```python
from build123d import *

# Parameters (mm, degrees)
SKETCH1_R             = 1.95
BOSS_EXTRUDE1_DEPTH   = 6
M2_TAPPED_HOLE2_D     = 1.6
M2_TAPPED_HOLE2_DEPTH = 6
M2_TAPPED_HOLE2_TIP   = 572.957422794


with BuildPart() as part:
    # Sketch1 → Boss-Extrude1 (new body)
    with BuildSketch(Plane(origin=(0, 0, 0), x_dir=(1, 0, 0), z_dir=(0, 1, 0))):
        Polygon((-6.315, 5.815), (-5.815, 6.315), (5.815, 6.315), (6.315, 5.815), (6.315, -5.815), (5.815, -6.315), (-5.815, -6.315), (-6.315, -5.815), align=None)
        with Locations(Location((0, 0, 0), (0, 0, 270))):
            Circle(SKETCH1_R, mode=Mode.SUBTRACT)
    extrude(amount=BOSS_EXTRUDE1_DEPTH)

    # M2 Tapped Hole2
    with Locations(Plane(origin=(0, 6, 0), x_dir=(-1, 0, 0), z_dir=(0, 1, 0))):
        with Locations((4.25, -4.25), (-4.25, -4.25), (-4.25, 4.25), (4.25, 4.25)):
            Hole(M2_TAPPED_HOLE2_D / 2, depth=M2_TAPPED_HOLE2_DEPTH)
            with Locations((0, 0, -(M2_TAPPED_HOLE2_DEPTH + M2_TAPPED_HOLE2_TIP / 2))):  # 0.16° drill point
                Cone(0, M2_TAPPED_HOLE2_D / 2, M2_TAPPED_HOLE2_TIP, mode=Mode.SUBTRACT)


solid = part.part
```
Can you work these out from the model? Positions are in its coordinate system, mm. Round coordinates to 2 decimals unless told otherwise and drop trailing zeros. Loops run counter-clockwise (first coordinate to the right, second up) from the corner with the lowest first, then second, coordinate; pieces in that order, holes last. Notation, with made-up numbers: M 31,-25 L 66,-25 A26 cw 66,10 Z; hole C 66,67 d1. An arc over 180 degrees is marked long. Write item = value, one per line. Start each with the question number.
(1) Suppose I cut it at B-B on z = 0. Write out the boundary of the cut face in (x, y) (3 decimals).
(2) I need wall thicknesses on line 1 along X through (y, z) = (1.6, -4.25) (3 decimals); line 2 along X through (y, z) = (2.2, -4.75) (1 decimal). Which ranges of each line are inside material? Lowest first, please.
(3) Suppose I cut it at A-A on x = 0. Write out the boundary of the cut face in (y, z) (3 decimals).
(4) Suppose I cut it at C-C on y = 3.35. Write out the boundary of the cut face in (x, z) (3 decimals), plus the area to 3 significant figures.
(5) Suppose I cut it at D-D on z = -4.25. Write out the boundary of the cut face in (x, y) (3 decimals), plus the area to 3 significant figures.
(6) If we mould it in two halves opening along X, with no side actions, what happens to faces 1 (the face through (1.5, 0, -1.5)), 2 (the face through (-4.42, 2.96, -5.03)), 3 (the face through (6.315, 3, 0))? For each: released by +X, released by -X, zero draft, split by the parting line, or undercut.
Answer block:
q1.outline = M -6.315,0 L -1.95,0 L -1.95,6 L -6.315,6 Z; M 1.95,0 L 6.315,0 L 6.315,6 L 1.95,6 Z
q2.line_1 = -6.315 to -5.05, -3.45 to 3.45, 5.05 to 6.315
q2.line_2 = -6.3 to -4.9, -3.6 to 3.6, 4.9 to 6.3
q3.outline = M 0,-6.315 L 6,-6.315 L 6,-1.95 L 0,-1.95 Z; M 0,1.95 L 6,1.95 L 6,6.315 L 0,6.315 Z
q4.outline = M -6.315,-5.815 L -5.815,-6.315 L 5.815,-6.315 L 6.315,-5.815 L 6.315,5.815 L 5.815,6.315 L -5.815,6.315 L -6.315,5.815 Z; hole C -4.25,-4.25 d1.6; hole C -4.25,4.25 d1.6; hole C 0,0 d3.9; hole C 4.25,-4.25 d1.6; hole C 4.25,4.25 d1.6
q4.area = 139 mm²
q5.outline = M -6.315,0 L -5.05,0 L -5.05,6 L -6.315,6 Z; M -3.45,0 L 3.45,0 L 3.45,6 L -3.45,6 Z; M 5.05,0 L 6.315,0 L 6.315,6 L 5.05,6 Z
q5.area = 56.6 mm²
q6.face_1 = zero draft
q6.face_2 = undercut
q6.face_3 = released by +X
